```python
from build123d import *

# Parameters (mm, degrees)
BASE_BLOCK_DEPTH           = 60
BORE_SKETCH_R              = 18
HALF_BORE_CUT_DEPTH        = 21
TOP_SLOT_SKETCH_W          = 80
TOP_SLOT_SKETCH_H          = 15
TOP_SLOT_CUT_DEPTH         = 21
SIDE_POCKET_A_SKETCH_W     = 27
SIDE_POCKET_A_SKETCH_H     = 40
SIDE_POCKET_A_DEPTH        = 40
FRAME_INFILL_A_DEPTH       = 40
TRIANGLE_WINDOW_A_SKETCH_W = 30
TRIANGLE_WINDOW_A_SKETCH_H = 27
TRIANGLE_WINDOW_A_DEPTH    = 40
SIDE_POCKET_B_SKETCH_W     = 30
SIDE_POCKET_B_SKETCH_H     = 40
SIDE_POCKET_B_DEPTH        = 40
FRAME_INFILL_B_DEPTH       = 40
TRIANGLE_WINDOW_B_SKETCH_W = 30
TRIANGLE_WINDOW_B_SKETCH_H = 27
TRIANGLE_WINDOW_B_DEPTH    = 40


with BuildPart() as part:
    # Base Profile Sketch → Base Block (new body)
    with BuildSketch(Plane.XY):
        Polygon((-47.817836812, 0), (102.182163188, 0), (102.182163188, 30), (67.182163188, 30), (67.182163188, 80), (-12.817836812, 80), (-12.817836812, 30), (-47.817836812, 30), align=None)
    extrude(amount=-BASE_BLOCK_DEPTH)

    # Bore Sketch → Half Bore Cut (cut)
    with BuildSketch(Plane(origin=(0, 80, 0), x_dir=(1, 0, 0), z_dir=(0, 1, 0))):
        with Locations(Location((27.182163188, 30, 0), (0, 0, 180))):
            Circle(BORE_SKETCH_R)
    extrude(amount=-HALF_BORE_CUT_DEPTH, mode=Mode.SUBTRACT)

    # Top Slot Sketch → Top Slot Cut (cut)
    with BuildSketch(Plane(origin=(0, 80, 0), x_dir=(1, 0, 0), z_dir=(0, 1, 0))):
        with Locations((27.182163188, 30)):
            Rectangle(TOP_SLOT_SKETCH_W, TOP_SLOT_SKETCH_H)
    extrude(amount=-TOP_SLOT_CUT_DEPTH, mode=Mode.SUBTRACT)

    # Side Pocket A Sketch → Side Pocket A (cut)
    with BuildSketch(Plane(origin=(0, 30, 0), x_dir=(1, 0, 0), z_dir=(0, 1, 0))):
        with Locations((88.682163188, 30)):
            Rectangle(SIDE_POCKET_A_SKETCH_W, SIDE_POCKET_A_SKETCH_H)
    extrude(amount=-SIDE_POCKET_A_DEPTH, mode=Mode.SUBTRACT)

    # Frame Infill A Sketch → Frame Infill A (add)
    with BuildSketch(Plane.XY.offset(-50)):
        Polygon((75.182163188, 30), (102.182163188, 0), (75.182163188, 0), align=None)
    extrude(amount=FRAME_INFILL_A_DEPTH)

    # Triangle Window A Sketch → Triangle Window A (cut)
    with BuildSketch(Plane(origin=(56.454233805, 50.808810425, 0), x_dir=(0, 0, -1), z_dir=(0.7432941462471663, 0.6689647316224498, 0))):
        with Locations((30, -46.495391232)):
            Rectangle(TRIANGLE_WINDOW_A_SKETCH_W, TRIANGLE_WINDOW_A_SKETCH_H)
    extrude(amount=-TRIANGLE_WINDOW_A_DEPTH, mode=Mode.SUBTRACT)

    # Side Pocket B Sketch → Side Pocket B (cut)
    with BuildSketch(Plane(origin=(0, 30, 0), x_dir=(1, 0, 0), z_dir=(0, 1, 0))):
        with Locations((-32.817836812, 30)):
            Rectangle(SIDE_POCKET_B_SKETCH_W, SIDE_POCKET_B_SKETCH_H)
    extrude(amount=-SIDE_POCKET_B_DEPTH, mode=Mode.SUBTRACT)

    # Frame Infill B Sketch → Frame Infill B (add)
    with BuildSketch(Plane.XY.offset(-50)):
        Polygon((-47.817836812, 0), (-17.817836812, 30), (-17.817836812, 0), align=None)
    extrude(amount=FRAME_INFILL_B_DEPTH)

    # Triangle Window B Sketch → Triangle Window B (cut)
    with BuildSketch(Plane(origin=(-23.908918406, 23.908918406, 0), x_dir=(0, 0, 1), z_dir=(-0.7071067811865476, 0.7071067811865476, 0))):
        with Locations((-30, -9.8859098)):
            Rectangle(TRIANGLE_WINDOW_B_SKETCH_W, TRIANGLE_WINDOW_B_SKETCH_H)
    extrude(amount=-TRIANGLE_WINDOW_B_DEPTH, mode=Mode.SUBTRACT)


solid = part.part
```
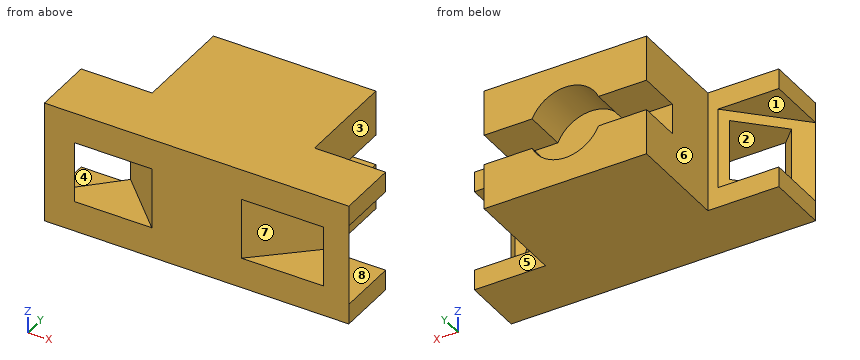
Model file for the job. Use its own axes, mm. Face numbers are marked on the shaded views. A direction names the side the tool comes from. Give positions to 0.01 mm unless a question says otherwise; leave off trailing zeros. Write each loop counter-clockwise with the first axis right and the second up, starting at its lowest first coordinate (ties: lowest second). Pieces come first, ordered by that corner, then holes. Notation, with made-up numbers: (60, 60) - (102, 60) arc R16 cw to (102, 87) - close; hole circle Ø4 at (-33.75, 63.5). An arc over 180 degrees is marked (long way). One line per question, with ' | ' between items. Start each with the question number.
(1) Slice it at A-A on y = 65. Write the cut outline in (x, z), plus the area to 3 significant figures.
(2) Slice it at C-C on z = -43. Write the cut outline in (x, y).
(3) Wall check: line 1 along Z through (x, y) = (77, 13); line 2 along X through (y, z) = (5.5, -40); line 3 along Y through (x, z) = (73, -12). Give the ranges that are in metal, low to high. Write a range as from..to.
(4) Pin check, flat tips, straight feed: P1, Ø3, axis at y = 19, z = -29.5, coming from the +X side; P2, Ø15, axis at y = 50.5, z = -39, coming from the +X side; P3, Ø12, axis at x = 87, z = -43.5, coming from the +Y side. Stop position of each tip, or through.
(5) 3-axis set-ups, long thin cutter, end or side, ignore diameter. For the marked faces 4, 5, 6, 7 and 8: which of +Z, -Z, +X, -X, +Y, -Y reach the whole face in a straight line?
(6) Slice it at D-D on z = -5.5. Write the cut outline in (x, y), plus the area to 3 significant figures.
(7) Two-plate mould, pull along X, no slides. Class the marked faces 1, 2 and 3: +X half, -X half, draft (parallel to the pull), parting line (faces both ways), or undercut.
(8) Slice it at B-B on x = -25. Write the cut outline in (y, z).
Results below:
1) outline: (-12.82, -60) - (67.18, -60) - (67.18, -37.5) - (43.55, -37.5) arc R18 cw to (10.82, -37.5) - (-12.82, -37.5) - close; (-12.82, -22.5) - (10.82, -22.5) arc R18 cw to (43.55, -22.5) - (67.18, -22.5) - (67.18, 0) - (-12.82, 0) - close | area: 3,110 mm^2
2) outline: (-47.82, 0) - (-33.07, 0) - (-40.45, 7.37) - close; (-21.35, 26.46) - (5.11, 0) - (49.32, 0) - (78.53, 26.28) - (75.18, 30) - (67.18, 30) - (67.18, 80) - (39.63, 80) - (39.63, 59) - (14.73, 59) - (14.73, 80) - (-12.82, 80) - (-12.82, 30) - (-17.82, 30) - close; (89.68, 0) - (102.18, 0) - (96.59, 6.21) - close
3) line 1: -60..-45, -15..0 | line 2: -42.32..-38.57, -0.39..55.43, 95.8..97.23 | line 3: 0..30
4) P1: x = 72.1 | P2: x = 67.18 | P3: y = 23.32
5) face 4: -X, +Y | face 5: +Z, -Z, +X, +Y | face 6: +Z, -Z, -X, +Y | face 7: -Y | face 8: +X, +Y
6) outline: (-47.82, 0) - (102.18, 0) - (102.18, 30) - (67.18, 30) - (67.18, 80) - (-12.82, 80) - (-12.82, 30) - (-47.82, 30) - close | area: 8,500 mm^2
7) face 1: draft | face 2: undercut | face 3: +X half
8) outline: (0, -60) - (30, -60) - (30, -50) - (22.82, -50) - (22.82, -45) - (0, -45) - close; (0, -15) - (22.82, -15) - (22.82, -10) - (30, -10) - (30, 0) - (0, 0) - close
